```python
from build123d import *

# Parameters (mm, degrees)
SKETCH_1_W          = 570
SKETCH_1_H          = 545
SKETCH_1_W_2        = 470
SKETCH_1_H_2        = 445
EXTRUDE_1_DEPTH     = 50
SKETCH_2_W          = 470
SKETCH_2_H          = 50
EXTRUDE_2_DEPTH     = 50
SKETCH_3_W          = 50
SKETCH_3_H          = 50
EXTRUDE_3_DEPTH     = 50
SKETCH_4_W          = 470
SKETCH_4_H          = 50
CUT_EXTRUDE_1_DEPTH = 50
EXTRUDE_4_DEPTH     = 478
SKETCH_6_W          = 570
SKETCH_6_H          = 50
CUT_EXTRUDE_2_DEPTH = 76
SKETCH_7_W          = 50
SKETCH_7_H          = 545
EXTRUDE_5_DEPTH     = 50
SKETCH_8_W          = 50
SKETCH_8_H          = 545
CUT_EXTRUDE_3_DEPTH = 50
SKETCH_9_W          = 50
SKETCH_9_H          = 50
EXTRUDE_6_DEPTH     = 20
SKETCH_10_W         = 50
SKETCH_10_H         = 50
EXTRUDE_7_DEPTH     = 10
SKETCH_11_W         = 50
SKETCH_11_H         = 50
EXTRUDE_8_DEPTH     = 60
SKETCH_12_W         = 50
SKETCH_12_H         = 50
EXTRUDE_9_DEPTH     = 45


with BuildPart() as part:
    # 草图1 → 凸台-拉伸1 (new body)
    with BuildSketch(Plane.XY):
        with Locations((285, 272.5)):
            Rectangle(SKETCH_1_W, SKETCH_1_H)
        with Locations((285, 272.5)):
            Rectangle(SKETCH_1_W_2, SKETCH_1_H_2, mode=Mode.SUBTRACT)
    extrude(amount=EXTRUDE_1_DEPTH)

    # 草图2 → 凸台-拉伸2 (add)
    with BuildSketch(Plane(origin=(0, 0, 0), x_dir=(-1, 0, 0), z_dir=(0, 0, -1))):
        with Locations((-285, 315)):
            Rectangle(SKETCH_2_W, SKETCH_2_H)
    extrude(amount=-EXTRUDE_2_DEPTH)

    # 草图3 → 凸台-拉伸3 (add)
    with BuildSketch(Plane.XZ):
        with Locations((25, 25)):
            Rectangle(SKETCH_3_W, SKETCH_3_H)
        with Locations((545, 25)):
            Rectangle(SKETCH_3_W, SKETCH_3_H)
    extrude(amount=EXTRUDE_3_DEPTH)

    # 草图4 → 切除-拉伸1 (cut)
    with BuildSketch(Plane.XY.offset(50)):
        with Locations((285, 25)):
            Rectangle(SKETCH_4_W, SKETCH_4_H)
    extrude(amount=-CUT_EXTRUDE_1_DEPTH, mode=Mode.SUBTRACT)

    # 草图5 → 凸台-拉伸4 (add)
    with BuildSketch(Plane.ZY.offset(-520)):
        Polygon((50, -50), (0, -50), (0, 0), (50, 0), (50, -10.325702711), align=None)
    extrude(amount=EXTRUDE_4_DEPTH)

    # 草图6 → 切除-拉伸2 (cut)
    with BuildSketch(Plane.XY.offset(50)):
        with Locations((285, -25)):
            Rectangle(SKETCH_6_W, SKETCH_6_H)
    extrude(amount=-CUT_EXTRUDE_2_DEPTH, mode=Mode.SUBTRACT)

    # 草图7 → 凸台-拉伸5 (add)
    with BuildSketch(Plane.ZY):
        with Locations((25, 272.5)):
            Rectangle(SKETCH_7_W, SKETCH_7_H)
    extrude(amount=-EXTRUDE_5_DEPTH)

    # 草图8 → 切除-拉伸3 (cut)
    with BuildSketch(Plane.ZY):
        with Locations((25, 272.5)):
            Rectangle(SKETCH_8_W, SKETCH_8_H)
    extrude(amount=-CUT_EXTRUDE_3_DEPTH, mode=Mode.SUBTRACT)

    # 草图9 → 凸台-拉伸6 (add)
    with BuildSketch(Plane.ZY.offset(-50)):
        with Locations((25, 520)):
            Rectangle(SKETCH_9_W, SKETCH_9_H)
        with Locations((25, 315)):
            Rectangle(SKETCH_9_W, SKETCH_9_H)
    extrude(amount=EXTRUDE_6_DEPTH)

    # 草图10 → 凸台-拉伸7 (add)
    with BuildSketch(Plane.ZY.offset(-30)):
        with Locations((25, 520)):
            Rectangle(SKETCH_10_W, SKETCH_10_H)
        with Locations((25, 315)):
            Rectangle(SKETCH_10_W, SKETCH_10_H)
    extrude(amount=EXTRUDE_7_DEPTH)

    # 草图11 → 凸台-拉伸8 (add)
    with BuildSketch(Plane.XZ):
        with Locations((545, 25)):
            Rectangle(SKETCH_11_W, SKETCH_11_H)
    extrude(amount=EXTRUDE_8_DEPTH)

    # 草图12 → 凸台-拉伸9 (add)
    with BuildSketch(Plane.ZY.offset(-20)):
        with Locations((25, 520)):
            Rectangle(SKETCH_12_W, SKETCH_12_H)
        with Locations((25, 315)):
            Rectangle(SKETCH_12_W, SKETCH_12_H)
    extrude(amount=EXTRUDE_9_DEPTH)


solid = part.part
```
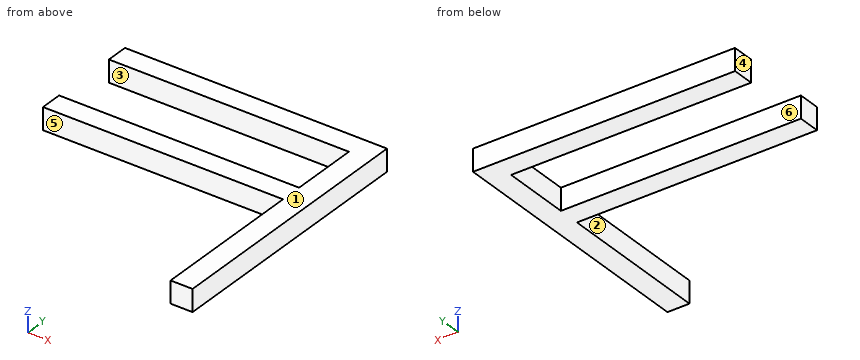
Geometry check sheet. Reference: the model listing, model coordinates, mm. Face numbers are marked on the shaded views. A direction names the side the tool comes from. Round coordinates to 2 decimals unless told otherwise and drop trailing zeros. Order: outer loops, then holes, each group sorted by start corner. A loop starts at its lowest first (then second) coordinate and runs counter-clockwise, first axis right, second up. Notation, with made-up numbers: (13, 6) - (26, 6) arc R28 ccw to (26, 41) - close; hole circle Ø2 at (-21, 88). An arc over 180 degrees is marked (long way). Use a Markdown table: item, result. Add a question column.
(1) Depth check by flat-ended pin: pin 1 (6 mm diameter, centred on x = 158, z = 38.5, fed in from -Y); pin 2 (5 mm diameter, centred on y = 87.5, z = 43, fed in from -X). Enter the tip coordinate at first touch or a pass-through.
(2) Tool access check on the marked faces 1, 2 and 3. Record the directions out of +Z, -Z, +X, -X, +Y, -Y that give a thin tool (end or side, any length) a straight path to the whole face; none if there is none.
(3) Sectioned sample at A-A, the plane x = 463. Enter the section's corners in (y, z), and give its area (3 significant figures).
(4) Sectioned sample at C-C, the plane y = 178.5. Enter the section's corners in (x, z).
(5) Sectioned sample at B-B, the plane z = 30. Enter the section's corners in (x, y).
(6) Release check for a two-part mould opening along Y. For the marked faces 4, 5 and 6 record: pulls with the +Y half, pulls with the -Y half, needs draft (parallel to the pull), parting line crosses it, or undercut.
(7) Material ranges on line 1 along Y through (x, z) = (166, 17); line 2 along X through (y, z) = (116, 23), recorded low to high. Write a range as [from, to].
Answers below:
| question | item | result |
|---|---|---|
| 1 | pin 1 | y = 290 |
| 1 | pin 2 | x = 520 |
| 2 | face 1 | +Z, +X, -X, +Y, -Y |
| 2 | face 2 | +Z, -Z, -X, -Y |
| 2 | face 3 | +Z, -Z, -X |
| 3 | outline | (290, 0) - (340, 0) - (340, 50) - (290, 50) - close; (495, 0) - (545, 0) - (545, 50) - (495, 50) - close |
| 3 | area | 5,000 mm² |
| 4 | outline | (520, 0) - (570, 0) - (570, 50) - (520, 50) - close |
| 5 | outline | (-25, 290) - (520, 290) - (520, -60) - (570, -60) - (570, 545) - (-25, 545) - (-25, 495) - (520, 495) - (520, 340) - (-25, 340) - close |
| 6 | face 4 | needs draft |
| 6 | face 5 | pulls with the -Y half |
| 6 | face 6 | undercut |
| 7 | line 1 | [290, 340], [495, 545] |
| 7 | line 2 | [520, 570] |
